Build history of the part. All positions in model axes, mm. Round coordinates to 2 decimals unless told otherwise and drop trailing zeros. Write each loop counter-clockwise with the first axis right and the second up, starting at its lowest first coordinate (ties: lowest second). Pieces come first, ordered by that corner, then holes.
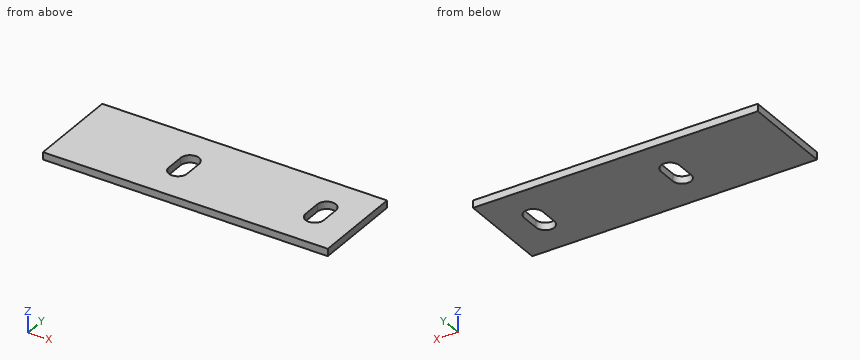
from build123d import *

# Parameters (mm, degrees)
BOSS_EXTRUDE1_DEPTH = 20


with BuildPart() as part:
    # Sketch1 → Boss-Extrude1 (new body)
    with BuildSketch(Plane.XY):
        Polygon((14040.331499194, 4658.160293083), (14040.331499194, 4408.160293083), (13265.233105958, 4408.160293083), (13265.233105872, 4658.160293083), align=None)
        with BuildLine():
            Line((13543.233105077, 4558.160293388), (13543.233105077, 4508.160293551))
            ThreePointArc((13543.233105077, 4508.160293551), (13568.233205921, 4483.160293631), (13593.233104917, 4508.160495399))
            Line((13593.233104917, 4508.160495399), (13593.233104917, 4558.159705819))
            ThreePointArc((13593.233104917, 4558.159705819), (13568.233398781, 4583.159999523), (13543.233105077, 4558.160293388))
        make_face(mode=Mode.SUBTRACT)
        with BuildLine():
            Line((13915.331499495, 4558.160293394), (13915.331499495, 4508.160293549))
            ThreePointArc((13915.331499495, 4508.160293549), (13940.331591876, 4483.160293859), (13965.331499344, 4508.160478461))
            Line((13965.331499344, 4508.160478461), (13965.331499344, 4558.159730803))
            ThreePointArc((13965.331499344, 4558.159730803), (13940.331780715, 4583.160012023), (13915.331499495, 4558.160293394))
        make_face(mode=Mode.SUBTRACT)
    extrude(amount=BOSS_EXTRUDE1_DEPTH)


solid = part.part
1) Slice it at A-A (y = 4526). Write the cut outline in (x, z).
Results:
outline: (13265.23, 0) - (13543.23, 0) - (13543.23, 20) - (13265.23, 20) - close; (13593.23, 0) - (13915.33, 0) - (13915.33, 20) - (13593.23, 20) - close; (13965.33, 0) - (14040.33, 0) - (14040.33, 20) - (13965.33, 20) - close
2) Wall check: L1, parallel to X at y = 4541.5, z = 10.25; L2, parallel to X at y = 4572, z = 10.25; L3, parallel to Y at x = 13574, z = 11. Give the ranges that are in metal, low to high.
Results:
L1: x = 13265.23 to 13543.23, 13593.23 to 13915.33, 13965.33 to 14040.33
L2: x = 13265.23 to 13547.41, 13589.05 to 13919.51, 13961.15 to 14040.33
L3: y = 4408.16 to 4483.83, 4582.49 to 4658.16
3) Slice it at B-B (z = 7). Write the cut outline in (x, y), plus the area to 3 significant figures.
Results:
outline: (13265.23, 4408.16) - (14040.33, 4408.16) - (14040.33, 4658.16) - (13265.23, 4658.16) - close; hole (13543.23, 4508.16) arc R25 ccw to (13593.23, 4508.16) - (13593.23, 4558.16) arc R25 ccw to (13543.23, 4558.16) - close; hole (13915.33, 4508.16) arc R25 ccw to (13965.33, 4508.16) - (13965.33, 4558.16) arc R25 ccw to (13915.33, 4558.16) - close
area: 185,000 mm2
